```python
from build123d import *

# Parameters (mm, degrees)
SKETCH_1_W                   = 100
SKETCH_1_H                   = 65
EXTRUDE_1_DEPTH              = 15
HOLE_WIZARD_M6_1_D           = 5
HOLE_WIZARD_M6_1_DEPTH       = 15
HOLE_WIZARD_M6_1_TIP         = 1.502151548
HOLE_WIZARD_M6_2_D           = 5
HOLE_WIZARD_M6_2_DEPTH       = 15
HOLE_WIZARD_M6_2_TIP         = 1.502151548
HOLE_WIZARD_M5_1_D           = 4.2
HOLE_WIZARD_M5_1_CSINK_D     = 5.05
HOLE_WIZARD_M5_1_CSINK_ANGLE = 90
HOLE_WIZARD_M6_3_D           = 5


with BuildPart() as part:
    # 草图1 → 凸台-拉伸1 (new body)
    with BuildSketch(Plane.XY):
        with Locations((50, 32.5)):
            Rectangle(SKETCH_1_W, SKETCH_1_H)
    extrude(amount=EXTRUDE_1_DEPTH)

    # M6 螺纹孔1
    with Locations(Plane(origin=(0, 65, 0), x_dir=(1, 0, 0), z_dir=(0, 1, 0))):
        with Locations((20, -7.5), (80, -7.5), (50, -7.5)):
            Hole(HOLE_WIZARD_M6_1_D / 2, depth=HOLE_WIZARD_M6_1_DEPTH)
            with Locations((0, 0, -(HOLE_WIZARD_M6_1_DEPTH + HOLE_WIZARD_M6_1_TIP / 2))):  # 118° drill point
                Cone(0, HOLE_WIZARD_M6_1_D / 2, HOLE_WIZARD_M6_1_TIP, mode=Mode.SUBTRACT)

    # M6 螺纹孔2
    with Locations(Plane(origin=(0, 0, 0), x_dir=(-1, 0, 0), z_dir=(0, -1, 0))):
        with Locations((-80, -7.5), (-50, -7.5), (-20, -7.5)):
            Hole(HOLE_WIZARD_M6_2_D / 2, depth=HOLE_WIZARD_M6_2_DEPTH)
            with Locations((0, 0, -(HOLE_WIZARD_M6_2_DEPTH + HOLE_WIZARD_M6_2_TIP / 2))):  # 118° drill point
                Cone(0, HOLE_WIZARD_M6_2_D / 2, HOLE_WIZARD_M6_2_TIP, mode=Mode.SUBTRACT)

    # M5 螺纹孔1 (through all)
    with Locations(Plane(origin=(0, 0, 0), x_dir=(-1, 0, 0), z_dir=(0, 0, -1))):
        with Locations((-70, 51), (-30, 51)):
            CounterSinkHole(HOLE_WIZARD_M5_1_D / 2, HOLE_WIZARD_M5_1_CSINK_D / 2, counter_sink_angle=HOLE_WIZARD_M5_1_CSINK_ANGLE)

    # M6 螺纹孔3 (through all)
    with Locations(Plane(origin=(0, 0, 0), x_dir=(-1, 0, 0), z_dir=(0, 0, -1))):
        with Locations((-90, 55), (-10, 55), (-90, 17), (-10, 17)):
            Hole(HOLE_WIZARD_M6_3_D / 2)


solid = part.part
```
Part model, mm, in its own coordinate system. A direction names the side the tool comes from. Round coordinates to 2 decimals unless told otherwise and drop trailing zeros. Loops run counter-clockwise (first coordinate to the right, second up) from the corner with the lowest first, then second, coordinate; pieces in that order, holes last.
Item 1: Mould opens along Y. For faces 4 (the face through (87.5, 55.1, 7.6)), 5 (the face through (0, 32, 7)), 6 (the face through (50.4, 48.76, 7.67)) say: +Y half, -Y half, draft (parallel to the pull), parting line (faces both ways), or undercut.
Item 2: Drop flat-ended pins along their axis: P1, Ø4.5, axis at x = 90, y = 17, coming from the -Z side; P2, Ø4.5, axis at x = 20, z = 7.5, coming from the -Y side; P3, Ø3, axis at x = 20, z = 7.5, coming from the +Y side. Give the stop position or say it passes through.
Item 3: Drill centre lines: line 1 (X direction, y = 51, z = 11.5); line 2 (Z direction, x = 80, y = 60.75); line 3 (X direction, y = 19, z = 3). Where is each one in solid material? Low to high.
Item 4: Cut at D-D, the plane z = 1.75. Give the cut face in (x, y), then the cut area to 3 significant figures.
Item 5: 3-axis set-ups, long thin cutter, end or side, ignore diameter. For faces 1 (the face through (22.5, 57.4, 7.4)), 2 (the face through (52.31, 7.6, 8.46)), 3 (the face through (49, 0, 4)): which of +Z, -Z, +X, -X, +Y, -Y reach the whole face in a straight line?
Item 6: Cut at B-B, the plane y = 51. Give the cut face in (x, z) (3 decimals).
Item 7: Cut at A-A, the plane x = 70. Give the cut face in (y, z) (3 decimals).
Item 8: Cut at C-C, the plane x = 90. Give the cut face in (y, z).
A:
1. face 4: undercut
1. face 5: draft
1. face 6: +Y half
2. P1: passes through
2. P2: stops at y = 15.15
2. P3: stops at y = 49.4
3. line 1: x = 0 to 27.9, 32.1 to 67.9, 72.1 to 100
3. line 2: z = 0 to 5, 10 to 15
3. line 3: x = 0 to 8.5, 11.5 to 88.5, 91.5 to 100
4. outline: (0, 0) - (100, 0) - (100, 65) - (0, 65) - close; hole circle Ø5 at (10, 17); hole circle Ø5 at (10, 55); hole circle Ø4.2 at (30, 51); hole circle Ø4.2 at (70, 51); hole circle Ø5 at (90, 17); hole circle Ø5 at (90, 55)
4. area: 6,390 mm2
5. face 1: +Y
5. face 2: -Y
5. face 3: +Z, -Z, +X, -X, -Y
6. outline: (0, 0) - (27.475, 0) - (27.9, 0.425) - (27.9, 15) - (0, 15) - close; (32.1, 0.425) - (32.525, 0) - (67.475, 0) - (67.9, 0.425) - (67.9, 15) - (32.1, 15) - close; (72.1, 0.425) - (72.525, 0) - (100, 0) - (100, 15) - (72.1, 15) - close; hole circle Ø5 at (20, 7.5); hole circle Ø5 at (50, 7.5); hole circle Ø5 at (80, 7.5)
7. outline: (0, 0) - (48.475, 0) - (48.9, 0.425) - (48.9, 15) - (0, 15) - close; (53.1, 0.425) - (53.525, 0) - (65, 0) - (65, 15) - (53.1, 15) - close
8. outline: (0, 0) - (14.5, 0) - (14.5, 15) - (0, 15) - close; (19.5, 0) - (52.5, 0) - (52.5, 15) - (19.5, 15) - close; (57.5, 0) - (65, 0) - (65, 15) - (57.5, 15) - close
